CAD build for the part. Positions are in the model's coordinates, mm. A direction names the side the tool comes from. Coordinates: 2 decimals unless noted, no trailing zeros. Loops run counter-clockwise (first coordinate to the right, second up) from the corner with the lowest first, then second, coordinate; pieces in that order, holes last. Notation, with made-up numbers: (-11, 44) - (45, 44) arc R32 ccw to (45, 81) - close; hole circle Ø4 at (38, 64.5). An arc over 180 degrees is marked (long way). Put each result on its own line as item: value.
```python
from build123d import *

# Parameters (mm, degrees)
EXTRUDE_THIN1_DEPTH = 1116
SKETCH2_W           = 42
SKETCH2_H           = 50
CUT_EXTRUDE1_DEPTH  = 1118.432772027
CUT_EXTRUDE2_DEPTH  = 10
LPATTERN1_COUNT     = 2
LPATTERN1_PITCH     = 430
LPATTERN2_COUNT     = 2
LPATTERN2_PITCH     = 430


with BuildPart() as part:
    # Sketch1 → Extrude-Thin1 (new body)
    with BuildSketch(Plane.XY):
        with BuildLine():
            Line((40, 0), (8, 0))
            ThreePointArc((8, 0), (2.343145751, 2.343145751), (0, 8))
            Line((0, 8), (0, 40))
            Line((0, 40), (4, 40))
            Line((4, 40), (4, 8))
            ThreePointArc((4, 8), (5.171572875, 5.171572875), (8, 4))
            Line((8, 4), (40, 4))
            Line((40, 4), (40, 0))
        make_face()
    extrude(amount=EXTRUDE_THIN1_DEPTH)

    # Sketch2 → Cut-Extrude1 (cut, through all)
    with BuildSketch(Plane(origin=(40, 0, 0), x_dir=(0, 0, -1), z_dir=(1, 0, 0))):
        with Locations((-280, 29)):
            Rectangle(SKETCH2_W, SKETCH2_H)
        with Locations((-836, 29)):
            Rectangle(SKETCH2_W, SKETCH2_H)
    extrude(amount=-CUT_EXTRUDE1_DEPTH, mode=Mode.SUBTRACT)

    # Sketch3 → Cut-Extrude2 (cut)
    with BuildSketch(Plane(origin=(0, 4, 0), x_dir=(1, 0, 0), z_dir=(0, 1, 0))):
        with BuildLine():
            Line((32, -551), (32, -565))
            ThreePointArc((32, -565), (25, -572), (18, -565))
            Line((18, -565), (18, -551))
            ThreePointArc((18, -551), (25, -544), (32, -551))
        make_face()
    cut_extrude2 = extrude(amount=-CUT_EXTRUDE2_DEPTH, mode=Mode.SUBTRACT)

    # LPattern1: Cut-Extrude2 ×2
    with Locations(*[(0, 0, -i * LPATTERN1_PITCH) for i in range(1, LPATTERN1_COUNT)]):
        add(cut_extrude2, mode=Mode.SUBTRACT)

    # LPattern2: Cut-Extrude2 ×2
    with Locations(*[(0, 0, i * LPATTERN2_PITCH) for i in range(1, LPATTERN2_COUNT)]):
        add(cut_extrude2, mode=Mode.SUBTRACT)


solid = part.part
```
Q1. Pin check, flat tips, straight feed: pin 1 Ø2 at (y, z) = (3, 989.5) entering from -X; pin 2 Ø16 at (y, z) = (18.5, 146.5) entering from +X; pin 3 Ø10 at (x, y) = (10.5, 22) entering from +Z; pin 4 Ø2 at (y, z) = (2, 125) entering from -X (3 decimals). Stop position of each tip, or through.
Determined:
pin 1: x = 1.07
pin 2: x = 4
pin 3: through
pin 4: x = 1.755
Q2. Slice it at B-B, the plane y = 19. Give the cut face in (x, z).
Determined:
outline: (0, 0) - (4, 0) - (4, 259) - (0, 259) - close; (0, 301) - (4, 301) - (4, 815) - (0, 815) - close; (0, 857) - (4, 857) - (4, 1116) - (0, 1116) - close
Q3. Tool access for faces 1 (the flat face through (11.2, 3.8, 1116)), 2 (the flat face through (4, 24, 128)): list every direction of +Z, -Z, +X, -X, +Y, -Y with a clear straight run to the whole face (end or side of a thin tool).
Determined:
face 1: +Z, +X, -X, +Y, -Y
face 2: +Z, -Z, +X, +Y
Q4. Wall check: L1, parallel to Y at x = 8, z = 443.5; L2, parallel to Y at x = 3.5, z = 769.5. Give the ranges that are in metal, low to high. Write a range as from..to.
Determined:
L1: 0..4
L2: 1.39..40
Q5. Slice it at A-A, the plane x = 25. Give the cut face in (y, z).
Determined:
outline: (0, 0) - (4, 0) - (4, 114) - (0, 114) - close; (0, 142) - (4, 142) - (4, 544) - (0, 544) - close; (0, 572) - (4, 572) - (4, 974) - (0, 974) - close; (0, 1002) - (4, 1002) - (4, 1116) - (0, 1116) - close
Q6. Slice it at C-C, the plane z = 505.5. Give the cut face in (x, y), then the cut area to 3 significant figures.
Determined:
outline: (0, 8) arc R8 ccw to (8, 0) - (40, 0) - (40, 4) - (8, 4) arc R4 cw to (4, 8) - (4, 40) - (0, 40) - close
area: 294 mm2
